Build history of the part. All positions in model axes, mm. A direction names the side the tool comes from. Round coordinates to 2 decimals unless told otherwise and drop trailing zeros. Write each loop counter-clockwise with the first axis right and the second up, starting at its lowest first coordinate (ties: lowest second). Pieces come first, ordered by that corner, then holes.
Item 1: Wall check: probe 1 along X at (y, z) = (31.8, 0) (3 decimals); probe 2 along Y at (x, z) = (-17.5, -6); probe 3 along Z at (x, y) = (6, 19). Give the ranges that are in metal, low to high.
Item 2: Mould opens along Z. For faces 4 (the flat face through (-2, 33.4, -16)), 5 (the cylindrical face through (-7.9, 15, 8.7)), 6 (the flat face through (-20, 33.4, 2)), 7 (the flat face through (-6, 38, 5)) say: +Z half, -Z half, draft (parallel to the pull), parting line (faces both ways), or undercut.
Item 3: Drop flat-ended pins along their axis: pin 1 Ø5 at (x, z) = (14, 18) entering from -Y; pin 2 Ø2 at (x, y) = (-6, 22.5) entering from +Z; pin 3 Ø7 at (x, z) = (0, -18) entering from +Y. Give the stop position or say it passes through.
Item 4: Band-saw the part on B-B, the plane y = 9. Write the cut outline in (x, z) (3 decimals).
Item 5: 3-axis set-ups, long thin cutter, end or side, ignore diameter. For faces 1 (the cylindrical face through (-7.509, 33.951, -23.846)), 2 (the flat face through (-6, 30, -11)), 3 (the flat face through (16, 33.4, 2)): which of +Z, -Z, +X, -X, +Y, -Y reach the whole face in a straight line?
Item 6: Band-saw the part on A-A, the plane z = 0. Count the separate pieces of the cut face and the enclosed holes in it, then the cut area to 3 significant figures.
```python
from build123d import *

# Parameters (mm, degrees)
G3_8_TAPPED_HOLE1_D                                 = 15.25
HOLE_SIZE_PER_SOCKET_HEAD_CAP_SCREW_TYP_D           = 4.5
HOLE_SIZE_PER_SOCKET_HEAD_CAP_SCREW_TYP_CBORE_D     = 8
HOLE_SIZE_PER_SOCKET_HEAD_CAP_SCREW_TYP_CBORE_DEPTH = 4.6
CHAMFER1_SIZE                                       = 0.5


with BuildPart() as part:
    # Sketch1 → Revolve1 (revolve)
    with BuildSketch(Plane.XY, mode=Mode.PRIVATE) as revolve1_sk:
        Polygon((0, 38), (-25, 38), (-25, 30), (-11.75, 30), (-11.75, 0), (0, 0), align=None)
    revolve(revolve1_sk.sketch.rotate(Axis((0, 0, 0), (0, 1, 0)), 270), axis=Axis((0, 0, 0), (0, 1, 0)))

    # G3/8 Tapped Hole1 (through all)
    with Locations(Plane.ZX.offset(38)):
        with Locations((0, 0)):
            Hole(G3_8_TAPPED_HOLE1_D / 2)

    # Hole Size (per socket head cap screw type)1 (through all)
    with Locations(Plane(origin=(0, 38, -18), x_dir=(0, 0, 1), z_dir=(0, 1, 0))):
        with Locations((0, 0), (18, -18), (18, 18), (36, 0)):
            CounterBoreHole(HOLE_SIZE_PER_SOCKET_HEAD_CAP_SCREW_TYP_D / 2, HOLE_SIZE_PER_SOCKET_HEAD_CAP_SCREW_TYP_CBORE_D / 2, HOLE_SIZE_PER_SOCKET_HEAD_CAP_SCREW_TYP_CBORE_DEPTH)

    # Chamfer1
    chamfer1_edges = [part.edges().sort_by_distance(p)[0] for p in [
        (0, 0, 11.75),
        (0, 30, 25),
        (0, 38, 25),
    ]]
    chamfer(chamfer1_edges, length=CHAMFER1_SIZE)


solid = part.part
```
Results:
1. probe 1: x = -25 to -20.25, -15.75 to -7.625, 7.625 to 15.75, 20.25 to 25
1. probe 2: y = 30 to 38
1. probe 3: z = -10.1 to -4.71, 4.71 to 10.1
2. face 4: undercut
2. face 5: parting line
2. face 6: undercut
2. face 7: draft
3. pin 1: stops at y = 30
3. pin 2: stops at z = 10.63
3. pin 3: stops at y = 33.4
4. outline: circle Ø23.5 at (0, 0); hole circle Ø15.25 at (0, 0)
5. face 1: +Y, -Y
5. face 2: -Y
5. face 3: +Y
6. separate pieces: 4
6. enclosed holes: 0
6. area: 421 mm2
